Source: CAD feature listing. Evaluate the final solid. Frame: model axes, mm. A direction names the side the tool comes from. Coordinates: 2 decimals unless noted, no trailing zeros. Loops run counter-clockwise (first coordinate to the right, second up) from the corner with the lowest first, then second, coordinate; pieces in that order, holes last.
Item 1: Pin query (flat end, axial travel): pin 1 Ø1.5 at (x, y) = (-0.5, -0.5) entering from -Z; pin 2 Ø8 at (x, z) = (-4.5, 26) entering from -Y; pin 3 Ø1 at (x, z) = (-1.5, 21) entering from +Y. Return the tip coordinate at first contact, or that it passes through.
Item 2: Line query: probe 1 along Y at (x, z) = (2.25, 10); probe 2 along Y at (x, z) = (0, 7.25); probe 3 along Z at (x, y) = (4, 0.5). Output: solid intervals per line, ascending.
Item 3: Pull-direction query (Y, two-part tool) for faces 4 (the flat face through (-3, 3, 20)), 5 (the flat face through (0, 6.5, 10)), 6 (the cylindrical face through (-1.43, 0.45, 6.41)), 7 (the cylindrical face through (3.8, 1, 8.69)); classes: +Y half, -Y half, draft (parallel to the pull), parting line (faces both ways), or undercut.
Item 4: Reachability of faces 1 (the cylindrical face through (3.233, -1.341, 20.493)), 2 (the cylindrical face through (3.8, 1, 2.69)), 3 (the cylindrical face through (-0.867, -3.905, 25.31)) from +Z, -Z, +X, -X, +Y, -Y: full face, straight path, thin tool, end or side. Return the list, or none.
Item 5: Section query A-A, the plane y = 0. State how many separate pieces and enclosed holes the cut face has, then the cut area to 3 significant figures.
Item 6: Section query D-D, the plane z = 27.5. Return the cut outline in (x, y).
Item 7: Section query B-B, the plane z = 4. Return the cut outline in (x, y), then the cut area to 3 significant figures.
```python
from build123d import *

# Parameters (mm, degrees)
SKETCH_1_R                  = 7.5
EXTRUDE_1_DEPTH             = 30
SKETCH_2_R                  = 8.226284638
SKETCH_2_R_2                = 4
CUT_EXTRUDE_1_DEPTH         = 10
SKETCH_3_R                  = 1.5
CUT_EXTRUDE_2_DEPTH         = 13
SKETCH_4_R                  = 4.479492859
SKETCH_4_R_2                = 3.5
CUT_EXTRUDE_3_DEPTH         = 1
CHAMFER_1_SIZE              = 0.5
SKETCH_6_W                  = 1.65
SKETCH_6_H                  = 7.5
HOLE_WIZARD_M4_1_AT_2_COUNT = 2
HOLE_WIZARD_M4_1_AT_2_PITCH = 6
SKETCH_7_W                  = 26.910087363
SKETCH_7_H                  = 4.855614415
SKETCH_7_W_2                = 23.143582724
SKETCH_7_H_2                = 3.131190604
CUT_EXTRUDE_4_DEPTH         = 5


with BuildPart() as part:
    # 草图1 → 凸台-拉伸1 (new body)
    with BuildSketch(Plane.XY):
        Circle(SKETCH_1_R)
    extrude(amount=EXTRUDE_1_DEPTH)

    # 草图2 → 切除-拉伸1 (cut)
    with BuildSketch(Plane.XY.offset(30)):
        Circle(SKETCH_2_R)
        Circle(SKETCH_2_R_2, mode=Mode.SUBTRACT)
    extrude(amount=-CUT_EXTRUDE_1_DEPTH, mode=Mode.SUBTRACT)

    # 草图3 → 切除-拉伸2 (cut)
    with BuildSketch(Plane(origin=(0, 0, 0), x_dir=(-1, 0, 0), z_dir=(0, 0, -1))):
        Circle(SKETCH_3_R)
    extrude(amount=-CUT_EXTRUDE_2_DEPTH, mode=Mode.SUBTRACT)

    # 草图4 → 切除-拉伸3 (cut)
    with BuildSketch(Plane.XY.offset(20)):
        Circle(SKETCH_4_R)
        Circle(SKETCH_4_R_2, mode=Mode.SUBTRACT)
    extrude(amount=CUT_EXTRUDE_3_DEPTH, mode=Mode.SUBTRACT)

    # 倒角1
    chamfer_1_edges = [part.edges().sort_by_distance(p)[0] for p in [
        (-7.5, 0, 0),
        (-7.5, 0, 20),
        (-4, 0, 30),
    ]]
    chamfer(chamfer_1_edges, length=CHAMFER_1_SIZE)

    # 草图6 → M4 螺纹孔1 (revolve, cut)
    with BuildSketch(Plane(origin=(0, 0, 4), x_dir=(0, 0, 1), z_dir=(0, 1, 0))):
        with Locations((0.825, 3.75)):
            Rectangle(SKETCH_6_W, SKETCH_6_H)
    hole_wizard_m4_1 = revolve(axis=Axis((-6.35, 0, 4), (1, 0, 0)), mode=Mode.SUBTRACT)

    # M4 螺纹孔1 at 2: M4 螺纹孔1 ×2
    with Locations(*[(0, 0, i * HOLE_WIZARD_M4_1_AT_2_PITCH) for i in range(1, HOLE_WIZARD_M4_1_AT_2_COUNT)]):
        add(hole_wizard_m4_1, mode=Mode.SUBTRACT)

    # 草图7 → 切除-拉伸4 (cut, symmetric)
    with BuildSketch(Plane(origin=(0, 0, 0), x_dir=(0, 0, -1), z_dir=(1, 0, 0))):
        with Locations((-11.641911526, 8.927807208)):
            Rectangle(SKETCH_7_W, SKETCH_7_H)
        with Locations((-10.167075372, -8.065595302)):
            Rectangle(SKETCH_7_W_2, SKETCH_7_H_2)
    extrude(amount=CUT_EXTRUDE_4_DEPTH, both=True, mode=Mode.SUBTRACT)


solid = part.part
```
Verdict:
1. pin 1: stops at z = 13
1. pin 2: stops at y = -3.97
1. pin 3: stops at y = 3.87
2. probe 1: y = -6.5 to -1.65, 1.65 to 6.5
2. probe 2: y = -6.5 to -1.5, 1.5 to 6.5
2. probe 3: z = 0 to 2.43, 5.57 to 8.43, 11.57 to 20
3. face 4: draft
3. face 5: +Y half
3. face 6: undercut
3. face 7: undercut
4. face 1: none
4. face 2: +X
4. face 3: +Z
5. separate pieces: 3
5. enclosed holes: 0
5. area: 300 mm2
6. outline: circle Ø8 at (0, 0)
7. outline: (-3.74, -6.5) - (3.74, -6.5) arc R7.5 ccw to (7.32, -1.65) - (0, -1.65) - (0, -1.5) arc R1.5 cw to (0, 1.5) - (0, 1.65) - (7.32, 1.65) arc R7.5 ccw to (3.74, 6.5) - (-3.74, 6.5) arc R7.5 ccw to start
7. area: 139 mm2
